Part model, mm, in its own coordinate system. A direction names the side the tool comes from. Round coordinates to 2 decimals unless told otherwise and drop trailing zeros. Order: outer loops, then holes, each group sorted by start corner. A loop starts at its lowest first (then second) coordinate and runs counter-clockwise, first axis right, second up. Notation, with made-up numbers: M 88,56 L 143,56 A12 cw 143,63 Z; hole C -34,57 d9. An arc over 180 degrees is marked long. One line per question, with ' | ' between items.
from build123d import *

# Parameters (mm, degrees)
EXTRUDE_1_DEPTH        = 12
HOLE_WIZARD_M5_1_D     = 4.2
HOLE_WIZARD_M5_1_DEPTH = 12.4
HOLE_WIZARD_M5_1_TIP   = 1.2618073
HOLE_WIZARD_M5_2_D     = 4.2
HOLE_WIZARD_M5_2_DEPTH = 12.4
HOLE_WIZARD_M5_2_TIP   = 1.2618073
CHAMFER_1_SIZE         = 2


with BuildPart() as part:
    # 草图1 → 凸台-拉伸1 (new body)
    with BuildSketch(Plane.XY):
        Polygon((0, 0), (0, -90), (-15, -90), (-70, -15), (-70, 0), align=None)
    extrude(amount=EXTRUDE_1_DEPTH)

    # M5 螺纹孔1
    with Locations(Plane(origin=(0, 0, 0), x_dir=(1, 0, 0), z_dir=(0, 1, 0))):
        with Locations((-60, -6), (-30, -6)):
            Hole(HOLE_WIZARD_M5_1_D / 2, depth=HOLE_WIZARD_M5_1_DEPTH)
            with Locations((0, 0, -(HOLE_WIZARD_M5_1_DEPTH + HOLE_WIZARD_M5_1_TIP / 2))):  # 118° drill point
                Cone(0, HOLE_WIZARD_M5_1_D / 2, HOLE_WIZARD_M5_1_TIP, mode=Mode.SUBTRACT)

    # M5 螺纹孔2
    with Locations(Plane(origin=(0, 0, 0), x_dir=(0, 0, -1), z_dir=(1, 0, 0))):
        with Locations((-6, -75), (-6, -25)):
            Hole(HOLE_WIZARD_M5_2_D / 2, depth=HOLE_WIZARD_M5_2_DEPTH)
            with Locations((0, 0, -(HOLE_WIZARD_M5_2_DEPTH + HOLE_WIZARD_M5_2_TIP / 2))):  # 118° drill point
                Cone(0, HOLE_WIZARD_M5_2_D / 2, HOLE_WIZARD_M5_2_TIP, mode=Mode.SUBTRACT)

    # 倒角1
    chamfer_1_edges = [part.edges().sort_by_distance(p)[0] for p in [
        (0, 0, 6),
    ]]
    chamfer(chamfer_1_edges, length=CHAMFER_1_SIZE)


solid = part.part
1) Saw through at C-C (x = -25). List the corners of the cut face in (y, z), plus the area to 3 significant figures.
The answers:
outline: M -76.36,0 L 0,0 L 0,12 L -76.36,12 Z | area: 916 mm²
2) Two-plate mould, pull along Z, no slides. Class faces 4 (the face through (-27, -34, 12)), 5 (the face through (-61.94, -6.29, 6.8)), 6 (the face through (-42.12, -53.02, 5.92)), 7 (the face through (-27, -34, 0)): released by +Z, released by -Z, zero draft, split by the parting line, or undercut.
The answers:
face 4: released by +Z | face 5: undercut | face 6: zero draft | face 7: released by -Z
3) Saw through at A-A (y = -5.5). List the corners of the cut face in (x, z), plus the area to 3 significant figures.
The answers:
outline: M -70,0 L 0,0 L 0,12 L -70,12 Z; hole C -60,6 d4.2; hole C -30,6 d4.2 | area: 812 mm²
4) Which spindle directions (+Z, -Z, +X, -X, +Y, -Y) get a long thin tool onto all of the face, cutting with end or side? Do faces 1 (the face through (-1, -1, 6)), 2 (the face through (-27.9, -6.29, 5.91)), 3 (the face through (-6.29, -23.23, 7.13)). Say none if no direction does.
The answers:
face 1: +Z, -Z, +X, +Y | face 2: +Y | face 3: +X
5) Drop flat-ended pins along their axis: pin 1 (6 mm diameter, centred on x = -60, z = 9.5, fed in from -Y); pin 2 (3 mm diameter, centred on y = -73.5, z = 2.5, fed in from +X); pin 3 (2.5 mm diameter, centred on y = -25, z = 6, fed in from -X); pin 4 (5 mm diameter, centred on x = -60, z = 6, fed in from -Y). Give the stop position or say it passes through.
The answers:
pin 1: stops at y = -32.73 | pin 2: stops at x = 0 | pin 3: stops at x = -63.58 | pin 4: stops at y = -32.05
6) Saw through at D-D (y = -16.5). List the corners of the cut face in (x, z), plus the area to 3 significant figures.
The answers:
outline: M -68.9,0 L 0,0 L 0,12 L -68.9,12 Z | area: 827 mm²
7) Saw through at B-B (z = 1.5). List the corners of the cut face in (x, y).
The answers:
outline: M -70,-15 L -15,-90 L 0,-90 L 0,-2 L -2,0 L -70,0 Z
8) Probe line 1 (Y direction, x = -6, z = 6); line 2 (Z direction, x = -60, y = -6); line 3 (X direction, y = -28, z = 6.5). List the from-to ranges inside material, lowest first. Write a range as [from, to].
The answers:
line 1: y = [-90, -77.1], [-72.9, -27.1], [-22.9, 0] | line 2: z = [0, 3.9], [8.1, 12] | line 3: x = [-60.47, 0]
